Verification items for the finished model (mm, model axes). Face numbers are marked on the shaded views. A direction names the side the tool comes from. Coordinates: 2 decimals unless noted, no trailing zeros. Order: outer loops, then holes, each group sorted by start corner. A loop starts at its lowest first (then second) coordinate and runs counter-clockwise, first axis right, second up. Notation, with made-up numbers: M 80.25,59 L 106.25,59 A22 cw 106.25,80 Z; hole C 36.25,48 d8. An arc over 180 degrees is marked long. Return JSON: item names as keys, results as strings. Group by question number.
Q1. Section check D-D, the plane z = -20. Enter the section's corners in (x, y).
Q2. Mould release check, pull along Y, two halves, no side actions. Record for the marked faces 1, 2, 3 and 4: pulls with the +Y half, pulls with the -Y half, needs draft (parallel to the pull), parting line crosses it, or undercut.
Q3. Thickness scan on probe 1 along Y at (x, z) = (8.75, 20); probe 2 along Y at (x, z) = (4, -20); probe 3 along Y at (x, z) = (1.85, 0). Record the ranges inside material, lowest first.
Q4. Section check B-B, the plane z = 0. Enter the section's corners in (x, y).
Q5. Section check A-A, the plane x = 8.5. Count the separate pieces of the cut face and the enclosed holes in it, then the cut area to 3 significant figures.
Q6. Access from +Z, -Z, +X, -X, +Y, -Y to the whole of each face (thin tool, end or side, straight path). Record for the marked faces 5 and 6.
Q7. Go/stop test with flat-tipped pins: pin 1 Ø5 at (y, z) = (10.5, 20) entering from +X; pin 2 Ø5 at (y, z) = (10, -21.5) entering from +X; pin 3 Ø6.5 at (y, z) = (12.5, 0) entering from -X. Record where each tip stops, or that it passes through.
Q8. Section check C-C, the plane y = -6. Enter the section's corners in (x, z), then the cut area to 3 significant figures.
from build123d import *

# Parameters (mm, degrees)
SKETCH1_W                                            = 60
SKETCH1_H                                            = 65
BOSS_EXTRUDE1_DEPTH                                  = 12
CBORE_FOR_M4_HEXAGON_SOCKET_HEAD_CAP_SCR_D           = 4.5
CBORE_FOR_M4_HEXAGON_SOCKET_HEAD_CAP_SCR_CBORE_D     = 8
CBORE_FOR_M4_HEXAGON_SOCKET_HEAD_CAP_SCR_CBORE_DEPTH = 4.6
CBORE_FOR_M5_HEXAGON_SOCKET_HEAD_CAP_SCR_D           = 5.5
CBORE_FOR_M5_HEXAGON_SOCKET_HEAD_CAP_SCR_CBORE_D     = 10
CBORE_FOR_M5_HEXAGON_SOCKET_HEAD_CAP_SCR_CBORE_DEPTH = 5.7
CHAMFER1_SIZE                                        = 2
F_5_0MM_BLIND_DOWEL_HOLE1_D                          = 5


with BuildPart() as part:
    # Sketch1 → Boss-Extrude1 (new body)
    with BuildSketch(Plane(origin=(0, 0, 0), x_dir=(0, 0, -1), z_dir=(1, 0, 0))):
        Rectangle(SKETCH1_W, SKETCH1_H)
    extrude(amount=BOSS_EXTRUDE1_DEPTH)

    # CBORE for M4 Hexagon socket head cap screws1 (through all)
    with Locations(Plane.ZY):
        with Locations((0, 12.5), (0, -22.5)):
            CounterBoreHole(CBORE_FOR_M4_HEXAGON_SOCKET_HEAD_CAP_SCR_D / 2, CBORE_FOR_M4_HEXAGON_SOCKET_HEAD_CAP_SCR_CBORE_D / 2, CBORE_FOR_M4_HEXAGON_SOCKET_HEAD_CAP_SCR_CBORE_DEPTH)

    # CBORE for M5 Hexagon socket head cap screws1 (through all)
    with Locations(Plane(origin=(12, 0, 0), x_dir=(0, 0, -1), z_dir=(1, 0, 0))):
        with Locations((-20, 10.5), (-20, -22.5), (20, -22.5), (20, 10.5)):
            CounterBoreHole(CBORE_FOR_M5_HEXAGON_SOCKET_HEAD_CAP_SCR_D / 2, CBORE_FOR_M5_HEXAGON_SOCKET_HEAD_CAP_SCR_CBORE_D / 2, CBORE_FOR_M5_HEXAGON_SOCKET_HEAD_CAP_SCR_CBORE_DEPTH)

    # Chamfer1
    chamfer1_edges = [part.edges().sort_by_distance(p)[0] for p in [
        (6, -32.5, -30),
        (6, -32.5, 30),
        (6, 32.5, 30),
        (6, 32.5, -30),
    ]]
    chamfer(chamfer1_edges, length=CHAMFER1_SIZE)

    # Ø5.0mm blind dowel hole1 (through all)
    with Locations(Plane(origin=(12, 0, 0), x_dir=(0, 0, -1), z_dir=(1, 0, 0))):
        with Locations((-20, -6), (20, -6)):
            Hole(F_5_0MM_BLIND_DOWEL_HOLE1_D / 2)


solid = part.part
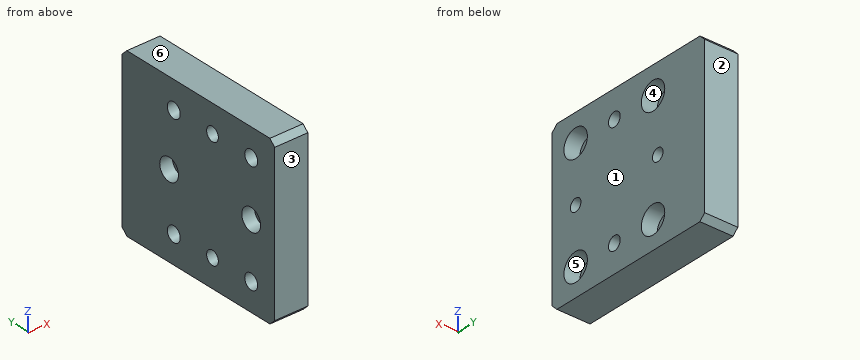
Numbers:
{
 "1": {"outline": "M 0,-32.5 L 12,-32.5 L 12,-27.5 L 6.3,-27.5 L 6.3,-25.25 L 0,-25.25 Z; M 0,-19.75 L 6.3,-19.75 L 6.3,-17.5 L 12,-17.5 L 12,-8.5 L 0,-8.5 Z; M 0,-3.5 L 12,-3.5 L 12,5.5 L 6.3,5.5 L 6.3,7.75 L 0,7.75 Z; M 0,13.25 L 6.3,13.25 L 6.3,15.5 L 12,15.5 L 12,32.5 L 0,32.5 Z"},
 "2": {"face 1": "needs draft", "face 2": "pulls with the +Y half", "face 3": "pulls with the -Y half", "face 4": "undercut"},
 "3": {"probe 1": "y = -32.5 to -27.5, -17.5 to -8.5, -3.5 to 5.5, 15.5 to 32.5", "probe 2": "y = -32.5 to -25.25, -19.75 to -8.5, -3.5 to 7.75, 13.25 to 32.5", "probe 3": "y = -32.5 to -26.5, -18.5 to 8.5, 16.5 to 32.5"},
 "4": {"outline": "M 0,-32.5 L 12,-32.5 L 12,-24.75 L 4.6,-24.75 L 4.6,-26.5 L 0,-26.5 Z; M 0,-18.5 L 4.6,-18.5 L 4.6,-20.25 L 12,-20.25 L 12,10.25 L 4.6,10.25 L 4.6,8.5 L 0,8.5 Z; M 0,16.5 L 4.6,16.5 L 4.6,14.75 L 12,14.75 L 12,32.5 L 0,32.5 Z"},
 "5": {"separate pieces": "1", "enclosed holes": "8", "area": "3,510 mm2"},
 "6": {"face 5": "+X", "face 6": "+Z, +X, -X, +Y, -Y"},
 "7": {"pin 1": "passes through", "pin 2": "stops at x = 6.3", "pin 3": "stops at x = 4.6"},
 "8": {"outline": "M 0,-30 L 12,-30 L 12,-22.5 L 0,-22.5 Z; M 0,-17.5 L 12,-17.5 L 12,17.5 L 0,17.5 Z; M 0,22.5 L 12,22.5 L 12,30 L 0,30 Z", "area": "600 mm2"}
}
